from build123d import *

# Parameters (mm, degrees)
SKETCH_2_R      = 0.85
EXTRUDE_1_DEPTH = 0.5
FILLET_1_R      = 1.266666667


with BuildPart() as part:
    # 草图2 → 凸台-拉伸1 (new, symmetric)
    with BuildSketch(Plane.XY):
        with BuildLine():
            Line((4.133871572, -9.701079585), (4.25, -7.793360231))
            ThreePointArc((4.25, -7.793360231), (0, 10.15), (-4.25, -7.793360231))
            Line((-4.25, -7.793360231), (-4.133871572, -9.701079585))
            ThreePointArc((-4.133871572, -9.701079585), (-3.705473422, -10.72960262), (-2.732214432, -11.271960018))
            Line((-2.732214432, -11.271960018), (-0.85, -11.603845206))
            Line((-0.85, -11.603845206), (-0.85, -7.803845206))
            ThreePointArc((-0.85, -7.803845206), (0, 7.85), (0.85, -7.803845206))
            Line((0.85, -7.803845206), (0.85, -11.603845206))
            Line((0.85, -11.603845206), (2.732214432, -11.271960018))
            ThreePointArc((2.732214432, -11.271960018), (3.705473422, -10.72960262), (4.133871572, -9.701079585))
        make_face()
        with Locations((2.55, -9.410632285)):
            Circle(SKETCH_2_R, mode=Mode.SUBTRACT)
        with Locations(Location((-2.55, -9.410632285, 0), (0, 0, 180))):
            Circle(SKETCH_2_R, mode=Mode.SUBTRACT)
    extrude(amount=EXTRUDE_1_DEPTH, both=True)

    # 圆角1
    fillet_1_edges = [part.edges().sort_by_distance(p)[0] for p in [
        (-4.25, -7.793360231, 0),
        (4.25, -7.793360231, 0),
    ]]
    fillet(fillet_1_edges, radius=FILLET_1_R)


solid = part.part
Check sheet for the modelled part. Datum: model origin and axes. Units: mm. A direction names the side the tool comes from. Give positions to 0.01 mm unless a question says otherwise; leave off trailing zeros. Write each loop counter-clockwise with the first axis right and the second up, starting at its lowest first coordinate (ties: lowest second). Pieces come first, ordered by that corner, then holes. Notation, with made-up numbers: (-12.75, 76.5) -> (-0.75, 76.5) arc R17 ccw to (-0.75, 100.5) -> close; hole circle Ø7 at (36, -17.75). An arc over 180 degrees is marked (long way). One line per item, written item: value. Start each with the question number.
Item 1: Section check A-A on y = 5.5. Record the cut outline in (x, z), then the cut area to 3 significant figures.
Item 2: Section check B-B on x = 7.5. Record the cut outline in (y, z).
Item 3: Tool access check on faces 4 (the flat face through (4.17, -9.1, 0.01)), 5 (the flat face through (-0.85, -10, 0)). Record the directions out of +Z, -Z, +X, -X, +Y, -Y that give a thin tool (end or side, any length) a straight path to the whole face; none if there is none.
Item 4: Material ranges on probe 1 along Y at (x, z) = (-3, -0.05); probe 2 along X at (y, z) = (-9.25, -0.25); probe 3 along Y at (x, z) = (-6.25, 0.4), recorded low to high. Write a range as from..to.
Item 5: Section check D-D on x = 0. Record the cut outline in (y, z), then the cut area to 3 significant figures.
Item 6: Draft check along Y on faces 1 (the flat face through (0.85, -10, 0)), 2 (the cylindrical face through (0.346, 10.144, 0.007)), 3 (the cylindrical face through (-0.333, 7.843, 0.007)). Enter one of: +Y half, -Y half, draft (parallel to the pull), parting line (faces both ways), or undercut.
Item 7: Section check C-C on z = 0. State how many separate pieces and enclosed holes the cut face has, then the cut area to 3 significant figures.
Item 8: Gauge pin test, flat ends, axial feed: pin 1 (4 mm diameter, centred on x = -6.5, y = -2.5, fed in from -Z); pin 2 (1.4 mm diameter, centred on x = -2.55, y = -9.41, fed in from -Z). Record the tip position at first contact, or that the pin passes through.
Results list:
1. outline: (-8.15, -0.5) -> (-5.6, -0.5) -> (-5.6, 0.5) -> (-8.15, 0.5) -> close; (5.6, -0.5) -> (8.15, -0.5) -> (8.15, 0.5) -> (5.6, 0.5) -> close
1. area: 5.11 mm²
2. outline: (-5.12, -0.5) -> (-2.32, -0.5) -> (-2.32, 0.5) -> (-5.12, 0.5) -> close; (2.32, -0.5) -> (6.47, -0.5) -> (6.47, 0.5) -> (2.32, 0.5) -> close
3. face 4: +Z, -Z, +X, -Y
3. face 5: +Z, -Z, -Y
4. probe 1: -11.2..-10.13, -8.69..-7.25, 7.25..9.66
4. probe 2: -4.16..-3.38, -1.72..-0.85, 0.85..1.72, 3.38..4.16
4. probe 3: -6.45..-4.75, 4.75..7.8
5. outline: (7.85, -0.5) -> (10.15, -0.5) -> (10.15, 0.5) -> (7.85, 0.5) -> close
5. area: 2.30 mm²
6. face 1: draft
6. face 2: parting line
6. face 3: undercut
7. separate pieces: 1
7. enclosed holes: 2
7. area: 101 mm²
8. pin 1: z = -0.5
8. pin 2: through
